from build123d import *

# Parameters (mm, degrees)
SKETCH2_R               = 4.5
CUT_EXTRUDE1_DEPTH      = 10
CUT_EXTRUDE1_DEPTH_BACK = 10
SKETCH3_R               = 1.5
CHAMFER1_SIZE           = 0.5


with BuildPart() as part:
    # Sweep1: sweep along a path in Sketch1
    with BuildLine(Plane.XY) as sweep1_path:
        Line((0, 0), (0, -18))
        ThreePointArc((0, -18), (4.246951673, -28.253048327), (14.5, -32.5))
        Line((14.5, -32.5), (305.5, -32.5))
        ThreePointArc((305.5, -32.5), (315.753048327, -28.253048327), (320, -18))
        Line((320, -18), (320, 0))
    # Sketch2 → Sweep1 (sweep)
    with BuildSketch(Plane(origin=(0, 0, 0), x_dir=(1, 0, 0), z_dir=(0, 1, 0))):
        Circle(SKETCH2_R)
    sweep(path=sweep1_path.line)

    # Sketch3 → Cut-Extrude1 (cut, two sides: drawn at the far end of the back side and taken through both)
    with BuildSketch(Plane.XY.offset(-CUT_EXTRUDE1_DEPTH_BACK)):
        with Locations(Location((320, -3, 0), (0, 0, 180))):
            Circle(SKETCH3_R)
        with Locations(Location((0, -3, 0), (0, 0, 180))):
            Circle(SKETCH3_R)
    extrude(amount=CUT_EXTRUDE1_DEPTH + CUT_EXTRUDE1_DEPTH_BACK, mode=Mode.SUBTRACT)

    # Chamfer1
    chamfer1_edges = [part.edges().sort_by_distance(p)[0] for p in [
        (-4.5, 0, 0),
        (324.5, 0, 0),
    ]]
    chamfer(chamfer1_edges, length=CHAMFER1_SIZE)


solid = part.part
Here's how the part is built. I have some questions about the finished solid (model axes, mm). A direction names the side the tool comes from. Coordinates: 2 decimals unless noted, no trailing zeros. Order: outer loops, then holes, each group sorted by start corner. A loop starts at its lowest first (then second) coordinate and runs counter-clockwise, first axis right, second up.
Item 1: If we mould it in two halves opening along X, with no side actions, what happens to faces 1 (the face through (0, 0, 0)), 2 (the face through (315.84, -9.13, -1.72)), 3 (the face through (162.037, -28.208, 1.352))? For each: +X half, -X half, draft (parallel to the pull), parting line (faces both ways), or undercut.
Result sheet:
face 1: draft
face 2: undercut
face 3: undercut
Item 2: If we section it at B-B on x = 270: List the corners of the cut face in (y, z) for me.
Result sheet:
outline: circle Ø9 at (-32.5, 0)
Item 3: If we section it at A-A on z = 0: List the corners of the cut face in (x, y) for me.
Result sheet:
outline: (-4.5, -18) arc R19 ccw to (14.5, -37) - (305.5, -37) arc R19 ccw to (324.5, -18) - (324.5, -0.5) - (324, 0) - (316, 0) - (315.5, -0.5) - (315.5, -18) arc R10 cw to (305.5, -28) - (14.5, -28) arc R10 cw to (4.5, -18) - (4.5, -0.5) - (4, 0) - (-4, 0) - (-4.5, -0.5) - close; hole circle Ø3 at (0, -3); hole circle Ø3 at (320, -3)
Item 4: For faces 4 (the face through (320, 0, 0)), 5 (the face through (4.292, -9.372, 1.352)), which set-ups out of +Z, -Z, +X, -X, +Y, -Y let a thin tool reach every point of the face, with its end or its side?
Result sheet:
face 4: +Z, -Z, +X, -X, +Y
face 5: +Y
Item 5: For P1, Ø4, axis at y = -6, z = -2, coming from the +X side; P2, Ø4, axis at y = -5, z = 3, coming from the +X side; P3, Ø3, axis at y = -31, z = 3.5, coming from the +X side; P4, Ø2, axis at x = 35, z = 1, coming from the +Y side, each with a flat end and sliding along its axis, tell me the tip position at first contact or that it passes through.
Result sheet:
P1: stops at x = 324.5
P2: stops at x = 324.39
P3: stops at x = 319.34
P4: stops at y = -28
Item 6: I need wall thicknesses on line 1 (X direction, y = -3, z = -0.5); line 2 (X direction, y = -3, z = -0.75); line 3 (Y direction, x = 0, z = -0.5). Which ranges of each line are inside material? Lowest first, please.
Result sheet:
line 1: x = -4.47 to -1.5, 1.5 to 4.47, 315.53 to 318.5, 321.5 to 324.47
line 2: x = -4.44 to -1.5, 1.5 to 4.44, 315.56 to 318.5, 321.5 to 324.44
line 3: y = -30.23 to -4.5, -1.5 to 0
